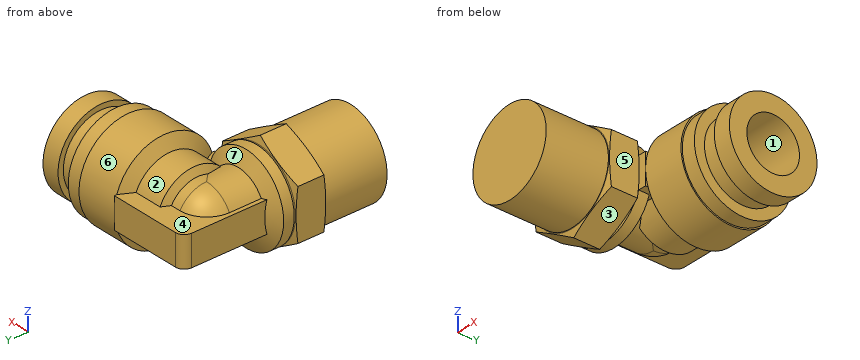
```python
from build123d import *

# Parameters (mm, degrees)
BOSS_EXTRUDE1_DEPTH      = 1.75
BOSS_EXTRUDE1_DEPTH_BACK = 1.75
SKETCH3_R                = 23.447488612
CUT_EXTRUDE1_DEPTH       = 3.4
HOLE1_D                  = 6
HOLE1_DEPTH              = 13.6


with BuildPart() as part:
    # Sketch1 → Revolve1 (revolve)
    with BuildSketch(Plane.XY, mode=Mode.PRIVATE) as revolve1_sk:
        Polygon((0, -3.1), (-4.864, -3.1), (-4.864, 4), (-4.95, 4), (-8, 4.817245037), (-8, 6.582754963), (-4.95, 7.4), (-3.3, 7.4), (-3.3, 7.6), (-5, 7.6), (-5, 8.803974596), (-3.5, 9.67), (-3.5, 13.3), (0, 13.3), align=None)
    revolve(revolve1_sk.sketch.rotate(Axis((0, 13.3, 0), (0, -1, 0)), 180), axis=Axis((0, 13.3, 0), (0, -1, 0)))

    # Sketch2 → Boss-Extrude1 (add, two sides: drawn at the far end of the back side and taken through both)
    with BuildSketch(Plane.XY.offset(-BOSS_EXTRUDE1_DEPTH_BACK)):
        with BuildLine():
            Line((-3.5, 7.6), (5.6, 7.6))
            Line((5.6, 7.6), (5.6, 19))
            Line((5.6, 19), (-2.5, 19))
            ThreePointArc((-2.5, 19), (-3.207106781, 18.707106781), (-3.5, 18))
            Line((-3.5, 18), (-3.5, 7.6))
        make_face()
    extrude(amount=BOSS_EXTRUDE1_DEPTH + BOSS_EXTRUDE1_DEPTH_BACK)

    # Sketch3 → Cut-Extrude1 (cut)
    with BuildSketch(Plane(origin=(0, 7.4, 0), x_dir=(1, 0, 0), z_dir=(0, 1, 0))):
        Circle(SKETCH3_R)
        Polygon((-5, 2.886751346), (-5, -2.886751346), (0, -5.773502692), (5, -2.886751346), (5, 2.886751346), (0, 5.773502692), align=None, mode=Mode.SUBTRACT)
    extrude(amount=-CUT_EXTRUDE1_DEPTH, mode=Mode.SUBTRACT)

    # Sketch4 → Revolve2 (revolve)
    with BuildSketch(Plane.XY, mode=Mode.PRIVATE) as revolve2_sk:
        with BuildLine():
            Line((0, 16.8), (1.138119785, 16.8))
            Line((1.138119785, 16.8), (1.6, 17.6))
            Line((1.6, 17.6), (4.791709623, 17.6))
            Line((4.791709623, 17.6), (5.6, 19))
            Line((5.6, 19), (10.3, 19))
            Line((10.3, 19), (10.3, 18.85))
            Line((10.3, 18.85), (11.9, 18.85))
            Line((11.9, 18.85), (11.9, 17.7))
            Line((11.9, 17.7), (13.9, 17.7))
            Line((13.9, 17.7), (13.9, 18.3))
            Line((13.9, 18.3), (15.9, 18.3))
            Line((15.9, 18.3), (15.9, 13.3))
            Line((15.9, 13.3), (-3.5, 13.3))
            ThreePointArc((-3.5, 13.3), (-2.474873734, 15.774873734), (0, 16.8))
        make_face()
    revolve(revolve2_sk.sketch.rotate(Axis((15.9, 13.3, 0), (-1, 0, 0)), 270), axis=Axis((15.9, 13.3, 0), (-1, 0, 0)))

    # Hole1
    with Locations(Plane(origin=(15.9, 0, 0), x_dir=(0, 0, -1), z_dir=(1, 0, 0))):
        with Locations((0, 13.3)):
            Hole(HOLE1_D / 2, depth=HOLE1_DEPTH)


solid = part.part
```
For this review, take the finished solid that the model builds, in its own axes (mm). Face numbers are marked on the shaded views. A direction names the side the tool comes from. Coordinates: 2 decimals unless noted, no trailing zeros. Write each loop counter-clockwise with the first axis right and the second up, starting at its lowest first coordinate (ties: lowest second). Pieces come first, ordered by that corner, then holes.
(1) Wall thickness on probe 1 along Y at (x, z) = (10.75, 0); probe 2 along Y at (x, z) = (12.25, 0); probe 3 along Z at (x, y) = (0.25, 17.5): over which ranges is each line inside the solid? List them lowest first.
(2) Add section A-A on x = 7.25. Give the boundary of the cut face in (y, z), then the cut area to 3 significant figures.
(3) Add section B-B on y = 1.75. Give the boundary of the cut face in (x, z).
(4) Tool access review of the marked faces 4, 5, 6 and 7: name each direction out of +Z, -Z, +X, -X, +Y, -Y from which nothing blocks a thin tool from reaching the whole face with its end or side.
(5) For pin 1 Ø5.5 at (y, z) = (13.3, 0) entering from +X; pin 2 Ø12 at (x, y) = (13.5, 8) entering from +Z; pin 3 Ø6 at (x, z) = (12, 1.5) entering from -Y, all flat-tipped, find the tip position at first contact; note any pin that passes through.
(6) The part is to be moulded in two halves that separate along X. For the marked faces 1, 2 and 3, say which applies: +X half, -X half, draft (parallel to the pull), parting line (faces both ways), or undercut.
Answer sheet:
1. probe 1: y = 7.75 to 10.3, 16.3 to 18.85
1. probe 2: y = 8.9 to 10.3, 16.3 to 17.7
1. probe 3: z = -1.75 to 1.75
2. outline: circle Ø11.4 at (13.3, 0); hole circle Ø6 at (13.3, 0)
2. area: 73.8 mm2
3. outline: circle Ø9.73 at (0, 0)
4. face 4: +Z, -X, +Y
4. face 5: +Z, -Z, +X, -Y
4. face 6: +X
4. face 7: none
5. pin 1: stops at x = 2.3
5. pin 2: stops at z = 5.7
5. pin 3: stops at y = 7.6
6. face 1: draft
6. face 2: undercut
6. face 3: +X half
